The listing builds one solid part. Answer for the finished solid, in the listing's coordinates (mm). Face numbers are marked on the shaded views. Coordinates: 2 decimals unless noted, no trailing zeros. Loops run counter-clockwise (first coordinate to the right, second up) from the corner with the lowest first, then second, coordinate; pieces in that order, holes last. Notation, with made-up numbers: (53, 55) - (94, 55) arc R14 cw to (94, 78) - close; hole circle Ø10 at (30, -5.5). An arc over 180 degrees is marked (long way). Return JSON: item names as keys, results as strings. Group by question number.
1. Each of these flat-tipped pins is pushed along its axis until it touches: P1, Ø4, axis at x = 0, y = 6, coming from the -Z side; P2, Ø8, axis at x = 14, z = 0, coming from the +Y side; P3, Ø8, axis at x = -28, z = 0, coming from the -Y side; P4, Ø5, axis at x = 29, y = 5, coming from the -Z side. Where does it stop, or does it pass through?
2. Section D-D (z = -14) is taken. Write down the section's boundary in (x, y), and give its area (3 significant figures).
3. Find the intervals of material crossed by line 1 along Z through (x, y) = (0, 1.25); line 2 along Y through (x, z) = (0, 41.25); line 3 along Y through (x, z) = (-18.5, 7), in increasing order.
4. Section A-A (z = 0) is taken. State how many separate pieces and enclosed holes the cut face has, and give its area (3 significant figures).
5. The mould has two halves that part along X. Classify the marked faces 1, 2 and 3: pulls with the +X half, pulls with the -X half, needs draft (parallel to the pull), parting line crosses it, or undercut.
6. Section C-C (x = 15.5) is taken. Write down the section's boundary in (y, z).
```python
from build123d import *

# Parameters (mm, degrees)
CUT_EXTRUDE1_REACH     = 60.902
SKETCH2_R              = 2.5
M3_TAPPED_HOLE1_REACH  = 94.991
M3_TAPPED_HOLE1_BORE_R = 1.25


with BuildPart() as part:
    # Sketch1 → Revolve1 (revolve)
    with BuildSketch(Plane.XY, mode=Mode.PRIVATE) as revolve1_sk:
        Polygon((1.75, 0), (1.75, 2), (3.25, 3.5), (40, 3.5), (40, 8.5), (41.5, 8.5), (41.5, 0), align=None)
    revolve(revolve1_sk.sketch.rotate(Axis((0, 9.310126582, 0), (0, -1, 0)), 180), axis=Axis((0, 9.310126582, 0), (0, -1, 0)))

    # Sketch2 → Cut-Extrude1 (cut, up to next)
    with BuildSketch(Plane(origin=(0, 3.5, 0), x_dir=(1, 0, 0), z_dir=(0, 1, 0)), mode=Mode.PRIVATE) as cut_extrude1_sk1:
        with Locations(Location((0, 14, 0), (0, 0, 180))):
            Circle(SKETCH2_R)
    cut_extrude1_tool1 = extrude(cut_extrude1_sk1.sketch, amount=-CUT_EXTRUDE1_REACH, mode=Mode.PRIVATE) & part.part
    # Sketch2 → Cut-Extrude1 (cut, up to next)
    with BuildSketch(Plane(origin=(0, 3.5, 0), x_dir=(1, 0, 0), z_dir=(0, 1, 0)), mode=Mode.PRIVATE) as cut_extrude1_sk2:
        with Locations(Location((14, 0, 0), (0, 0, 180))):
            Circle(SKETCH2_R)
    cut_extrude1_tool2 = extrude(cut_extrude1_sk2.sketch, amount=-CUT_EXTRUDE1_REACH, mode=Mode.PRIVATE) & part.part
    # Sketch2 → Cut-Extrude1 (cut, up to next)
    with BuildSketch(Plane(origin=(0, 3.5, 0), x_dir=(1, 0, 0), z_dir=(0, 1, 0)), mode=Mode.PRIVATE) as cut_extrude1_sk3:
        with Locations(Location((0, 28, 0), (0, 0, 180))):
            Circle(SKETCH2_R)
    cut_extrude1_tool3 = extrude(cut_extrude1_sk3.sketch, amount=-CUT_EXTRUDE1_REACH, mode=Mode.PRIVATE) & part.part
    # Sketch2 → Cut-Extrude1 (cut, up to next)
    with BuildSketch(Plane(origin=(0, 3.5, 0), x_dir=(1, 0, 0), z_dir=(0, 1, 0)), mode=Mode.PRIVATE) as cut_extrude1_sk4:
        with Locations(Location((28, 0, 0), (0, 0, 180))):
            Circle(SKETCH2_R)
    cut_extrude1_tool4 = extrude(cut_extrude1_sk4.sketch, amount=-CUT_EXTRUDE1_REACH, mode=Mode.PRIVATE) & part.part
    # Sketch2 → Cut-Extrude1 (cut, up to next)
    with BuildSketch(Plane(origin=(0, 3.5, 0), x_dir=(1, 0, 0), z_dir=(0, 1, 0)), mode=Mode.PRIVATE) as cut_extrude1_sk5:
        with Locations(Location((0, -14, 0), (0, 0, 180))):
            Circle(SKETCH2_R)
    cut_extrude1_tool5 = extrude(cut_extrude1_sk5.sketch, amount=-CUT_EXTRUDE1_REACH, mode=Mode.PRIVATE) & part.part
    # Sketch2 → Cut-Extrude1 (cut, up to next)
    with BuildSketch(Plane(origin=(0, 3.5, 0), x_dir=(1, 0, 0), z_dir=(0, 1, 0)), mode=Mode.PRIVATE) as cut_extrude1_sk6:
        with Locations(Location((0, -28, 0), (0, 0, 180))):
            Circle(SKETCH2_R)
    cut_extrude1_tool6 = extrude(cut_extrude1_sk6.sketch, amount=-CUT_EXTRUDE1_REACH, mode=Mode.PRIVATE) & part.part
    # Sketch2 → Cut-Extrude1 (cut, up to next)
    with BuildSketch(Plane(origin=(0, 3.5, 0), x_dir=(1, 0, 0), z_dir=(0, 1, 0)), mode=Mode.PRIVATE) as cut_extrude1_sk7:
        with Locations(Location((-14, 0, 0), (0, 0, 180))):
            Circle(SKETCH2_R)
    cut_extrude1_tool7 = extrude(cut_extrude1_sk7.sketch, amount=-CUT_EXTRUDE1_REACH, mode=Mode.PRIVATE) & part.part
    # Sketch2 → Cut-Extrude1 (cut, up to next)
    with BuildSketch(Plane(origin=(0, 3.5, 0), x_dir=(1, 0, 0), z_dir=(0, 1, 0)), mode=Mode.PRIVATE) as cut_extrude1_sk8:
        with Locations(Location((-28, 0, 0), (0, 0, 180))):
            Circle(SKETCH2_R)
    cut_extrude1_tool8 = extrude(cut_extrude1_sk8.sketch, amount=-CUT_EXTRUDE1_REACH, mode=Mode.PRIVATE) & part.part
    add(cut_extrude1_tool1.solids().sort_by_distance((0, 3.5, -14))[0], mode=Mode.SUBTRACT)
    add(cut_extrude1_tool2.solids().sort_by_distance((14, 3.5, 0))[0], mode=Mode.SUBTRACT)
    add(cut_extrude1_tool3.solids().sort_by_distance((0, 3.5, -28))[0], mode=Mode.SUBTRACT)
    add(cut_extrude1_tool4.solids().sort_by_distance((28, 3.5, 0))[0], mode=Mode.SUBTRACT)
    add(cut_extrude1_tool5.solids().sort_by_distance((0, 3.5, 14))[0], mode=Mode.SUBTRACT)
    add(cut_extrude1_tool6.solids().sort_by_distance((0, 3.5, 28))[0], mode=Mode.SUBTRACT)
    add(cut_extrude1_tool7.solids().sort_by_distance((-14, 3.5, 0))[0], mode=Mode.SUBTRACT)
    add(cut_extrude1_tool8.solids().sort_by_distance((-28, 3.5, 0))[0], mode=Mode.SUBTRACT)

    # M3 Tapped Hole1 bore (on position points) → M3 Tapped Hole1 (cut, up to next)
    with BuildSketch(Plane(origin=(0, 6, 41.5), x_dir=(1, 0, 0), z_dir=(0, 0, 1)), mode=Mode.PRIVATE) as m3_tapped_hole1_sk1:
        Circle(M3_TAPPED_HOLE1_BORE_R)
    m3_tapped_hole1_tool1 = extrude(m3_tapped_hole1_sk1.sketch, amount=-M3_TAPPED_HOLE1_REACH, mode=Mode.PRIVATE) & part.part
    add(m3_tapped_hole1_tool1.solids().sort_by_distance((0, 6, 41.5))[0], mode=Mode.SUBTRACT)


solid = part.part
```
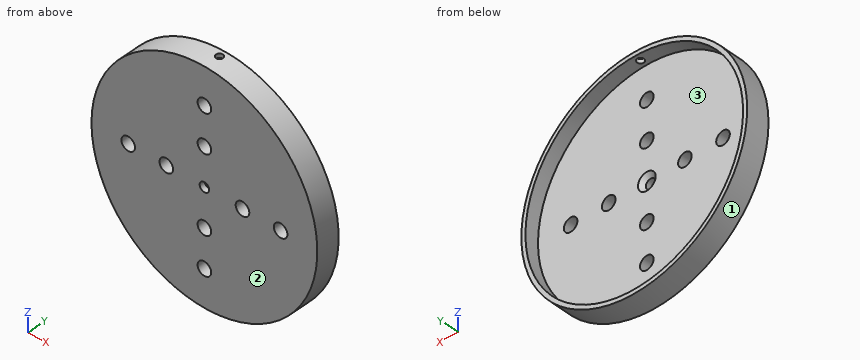
The answers:
{
 "1": {"P1": "stops at z = -41.5", "P2": "stops at y = 3.5", "P3": "stops at y = 0", "P4": "stops at z = -31.94"},
 "2": {"outline": "(-39.07, 0) - (-2.5, 0) - (-2.5, 3.5) - (-37.47, 3.5) - (-37.47, 8.5) - (-39.07, 8.5) - close; (2.5, 0) - (39.07, 0) - (39.07, 8.5) - (37.47, 8.5) - (37.47, 3.5) - (2.5, 3.5) - close", "area": "272 mm2"},
 "3": {"line 1": "z = -41.5 to -30.5, -25.5 to -16.5, -11.5 to -1.75, 1.75 to 11.5, 16.5 to 25.5, 30.5 to 41.5", "line 2": "y = 0 to 4.75, 7.25 to 8.5", "line 3": "y = 0 to 3.5"},
 "4": {"separate pieces": "6", "enclosed holes": "0", "area": "221 mm2"},
 "5": {"face 1": "parting line crosses it", "face 2": "needs draft", "face 3": "undercut"},
 "6": {"outline": "(0, -38.5) - (8.5, -38.5) - (8.5, -36.87) - (3.5, -36.87) - (3.5, -2) - (0, -2) - close; (0, 2) - (3.5, 2) - (3.5, 36.87) - (8.5, 36.87) - (8.5, 38.5) - (0, 38.5) - close"}
}
